Input: part model. Units: mm. Frame: model coordinates. Round coordinates to 2 decimals unless told otherwise and drop trailing zeros. Loops run counter-clockwise (first coordinate to the right, second up) from the corner with the lowest first, then second, coordinate; pieces in that order, holes last. Notation, with made-up numbers: (80.5, 63.25) - (93.5, 63.25) arc R30 cw to (93.5, 97.25) - close; hole circle Ø3 at (23.25, 16). An arc over 180 degrees is marked (long way). Use CSV: the item, a comma, the result in double quotes. Start each with the question number.
1. Pin query (flat end, axial travel): P1, Ø6, axis at x = 2377.93, z = -258.5, coming from the +Y side; P2, Ø4, axis at x = 2377.93, z = 228.5, coming from the +Y side; P3, Ø4, axis at y = 422.5, z = 229.5, coming from the -X side; P4, Ø1.5, axis at y = 424.5, z = -216.5, coming from the +X side. Return the tip coordinate at first contact, or that it passes through.
2. Cut plane A-A (z = -240). Return loops of the section in (x, y), and give its area (3 significant figures).
3. Material intervals for probe 1 along X at (y, z) = (422.5, 33.5); probe 2 along Y at (x, z) = (2389, 282); probe 3 along Y at (x, z) = (2378.5, 280.5), sorted ascending. Write a range as from..to.
```python
from build123d import *

# Parameters (mm, degrees)
MODEL_R             = 2.5
EXTRUDE_1_DEPTH     = 358.5
CUT_EXTRUDE_1_DEPTH = 2420.679144403
HOLE_WIZARD_M6_1_D  = 5


with BuildPart() as part:
    # Model → 凸台-拉伸1 (new, symmetric)
    with BuildSketch(Plane.XY):
        with BuildLine():
            Line((2390.427059452, 419.756797217), (2392.927059452, 419.756797217))
            Line((2392.927059452, 419.756797217), (2392.927059452, 415.406797217))
            Line((2392.927059452, 415.406797217), (2362.927059452, 415.406797217))
            Line((2362.927059452, 415.406797217), (2362.927059452, 419.756797217))
            Line((2362.927059452, 419.756797217), (2365.427059452, 419.756797217))
            Line((2365.427059452, 419.756797217), (2365.427059452, 417.706797217))
            Line((2365.427059452, 417.706797217), (2371.857059452, 417.706797217))
            ThreePointArc((2371.857059452, 417.706797217), (2373.727059452, 422.906797217), (2371.857059452, 428.106797217))
            Line((2371.857059452, 428.106797217), (2365.427059452, 428.106797217))
            Line((2365.427059452, 428.106797217), (2365.427059452, 426.056797217))
            Line((2365.427059452, 426.056797217), (2362.927059452, 426.056797217))
            Line((2362.927059452, 426.056797217), (2362.927059452, 430.406797217))
            Line((2362.927059452, 430.406797217), (2392.927059452, 430.406797217))
            Line((2392.927059452, 430.406797217), (2392.927059452, 426.056797217))
            Line((2392.927059452, 426.056797217), (2390.427059452, 426.056797217))
            Line((2390.427059452, 426.056797217), (2390.427059452, 428.106797217))
            Line((2390.427059452, 428.106797217), (2383.994799144, 428.106797217))
            ThreePointArc((2383.994799144, 428.106797217), (2382.127059452, 422.906797217), (2383.994799144, 417.706797217))
            Line((2383.994799144, 417.706797217), (2390.427059452, 417.706797217))
            Line((2390.427059452, 417.706797217), (2390.427059452, 419.756797217))
        make_face()
        with Locations((2377.927059452, 422.906797217)):
            Circle(MODEL_R, mode=Mode.SUBTRACT)
    extrude(amount=EXTRUDE_1_DEPTH, both=True)

    # 草图1 → 切除-拉伸1 (cut, through all)
    with BuildSketch(Plane(origin=(0, 430.406797217, 0), x_dir=(1, 0, 0), z_dir=(0, 1, 0))):
        Polygon((2362.927059452, 358.5), (2392.927059452, 328.5), (2392.927059452, 358.5), align=None)
        Polygon((2362.927059452, -358.5), (2392.927059452, -328.5), (2392.927059452, -358.5), align=None)
    extrude(amount=-CUT_EXTRUDE_1_DEPTH, mode=Mode.SUBTRACT)

    # M6 螺纹孔1 (through all)
    with Locations(Plane(origin=(0, 430.406797217, 0), x_dir=(1, 0, 0), z_dir=(0, 1, 0))):
        with Locations((2377.927059452, -258.5), (2377.927059452, -228.5), (2377.927059452, 228.5), (2377.927059452, 258.5)):
            Hole(HOLE_WIZARD_M6_1_D / 2)


solid = part.part
```
Established:
1,P1,"stops at y = 430.41"
1,P2,"passes through"
1,P3,"stops at x = 2373.36"
1,P4,"stops at x = 2382.47"
2,outline,"(2362.93, 415.41) - (2392.93, 415.41) - (2392.93, 419.76) - (2390.43, 419.76) - (2390.43, 417.71) - (2383.99, 417.71) arc R8.17 cw to (2383.99, 428.11) - (2390.43, 428.11) - (2390.43, 426.06) - (2392.93, 426.06) - (2392.93, 430.41) - (2362.93, 430.41) - (2362.93, 426.06) - (2365.43, 426.06) - (2365.43, 428.11) - (2371.86, 428.11) arc R8.16 cw to (2371.86, 417.71) - (2365.43, 417.71) - (2365.43, 419.76) - (2362.93, 419.76) - close; hole circle Ø5 at (2377.93, 422.91)"
2,area,"239 mm2"
3,probe 1,"x = 2373.72..2375.46, 2380.39..2382.14"
3,probe 2,"y = 415.41..417.71, 428.11..430.41"
3,probe 3,"y = 415.41..420.47, 425.34..430.41"
